Could you check a few things on this model? Use its own coordinates, in mm. Coordinates: 2 decimals unless noted, no trailing zeros. Write each loop counter-clockwise with the first axis right and the second up, starting at its lowest first coordinate (ties: lowest second). Pieces come first, ordered by that corner, then holes.
```python
from build123d import *

# Parameters (mm, degrees)
SKETCH_1_R          = 7.646875
EXTRUDE_555_DEPTH   = 17
SKETCH_2_OUTSIDE_W  = 129.344
SKETCH_2_OUTSIDE_H  = 133.304
SKETCH_2_OUTSIDE_R  = 13.5
CUT_EXTRUDE_1_DEPTH = 26.909162472
CUT_EXTRUDE_1_DRAFT = -60
CHAMFER_1_SIZE      = 0.294642857
SKETCH_9_OUTSIDE_W  = 89.946
SKETCH_9_OUTSIDE_H  = 93.906
SKETCH_9_OUTSIDE_R  = 12.15
CUT_EXTRUDE_7_DEPTH = 26.909162472
CUT_EXTRUDE_7_DRAFT = -45


with BuildPart() as part:
    # 草图1 → Extrude 555 (new body)
    with BuildSketch(Plane.XY):
        Polygon((0, 14.78), (-12.799855468, 7.39), (-12.799855468, -7.39), (0, -14.78), (12.799855468, -7.39), (12.799855468, 7.39), align=None)
        Circle(SKETCH_1_R, mode=Mode.SUBTRACT)
    extrude(amount=EXTRUDE_555_DEPTH)


with BuildPart() as cut_extrude_1_tool:
    # 草图2 outside → 切除-拉伸1 (with draft: the straight prism first)
    with BuildSketch(Plane(origin=(0, 0, 0), x_dir=(-1, 0, 0), z_dir=(0, 0, -1))):
        Rectangle(SKETCH_2_OUTSIDE_W, SKETCH_2_OUTSIDE_H)
        Circle(SKETCH_2_OUTSIDE_R, mode=Mode.SUBTRACT)
    extrude(amount=-CUT_EXTRUDE_1_DEPTH)
    # 切除-拉伸1: the draft: its side faces are tilted about the plane it starts from
    cut_extrude_1_sides = [cut_extrude_1_tool.faces().sort_by_distance(p)[0] for p in [
        (0, -66.652, 13.454581236),
        (-64.672, 0, 13.454581236),
        (0, 66.652, 13.454581236),
        (64.672, 0, 13.454581236),
        (13.5, 0, 13.454581236),
    ]]
    draft(cut_extrude_1_sides, Plane(origin=(0, 0, 0), x_dir=(-1, 0, 0), z_dir=(0, 0, -1)), CUT_EXTRUDE_1_DRAFT)


with BuildPart() as part_1:
    add(part.part)

    # 切除-拉伸1: cut by cut_extrude_1_tool
    add(cut_extrude_1_tool.part, mode=Mode.SUBTRACT)

    # 倒角1
    chamfer_1_edges = [part_1.edges().sort_by_distance(p)[0] for p in [
        (-7.646875, 0, 0),
    ]]
    chamfer(chamfer_1_edges, length=CHAMFER_1_SIZE)


with BuildPart() as cut_extrude_7_tool:
    # 草图9 outside → 切除-拉伸7 (with draft: the straight prism first)
    with BuildSketch(Plane.XY.offset(17)):
        Rectangle(SKETCH_9_OUTSIDE_W, SKETCH_9_OUTSIDE_H)
        Circle(SKETCH_9_OUTSIDE_R, mode=Mode.SUBTRACT)
    extrude(amount=-CUT_EXTRUDE_7_DEPTH)
    # 切除-拉伸7: the draft: its side faces are tilted about the plane it starts from
    cut_extrude_7_sides = [cut_extrude_7_tool.faces().sort_by_distance(p)[0] for p in [
        (0, -46.953, 3.545418764),
        (44.973, 0, 3.545418764),
        (0, 46.953, 3.545418764),
        (-44.973, 0, 3.545418764),
        (-12.15, 0, 3.545418764),
    ]]
    draft(cut_extrude_7_sides, Plane.XY.offset(17), CUT_EXTRUDE_7_DRAFT)


with BuildPart() as part_2:
    add(part_1.part)

    # 切除-拉伸7: cut by cut_extrude_7_tool
    add(cut_extrude_7_tool.part, mode=Mode.SUBTRACT)


solid = part_2.part
```
Item 1: If we mould it in two halves opening along Y, with no side actions, what happens to faces 1 (the flat face through (6.49, 11.033, 8.061)), 2 (the flat face through (-12.8, 0, 8)), 3 (the conical face through (-11.97, -6.96, 0.2)), 4 (the cylindrical face through (-5.636, 5.168, 8.53))? For each: released by +Y, released by -Y, zero draft, split by the parting line, or undercut.
Item 2: If I drill on line 1 along X through (y, z) = (-0.75, 4.5); line 2 along Y through (x, z) = (5.75, 11); line 3 along X through (y, z) = (1.5, 12), over which ranges is the centre line in solid material (lowest first)?
Item 3: Will this pin go through, and if not, where does the flat tip stop? pin 1 Ø1 at (x, z) = (6, 6.5) entering from +Y.
Item 4: I want a section at B-B, the plane z = 7.5. List the corners of the cut face in (x, y) for me.
Item 5: I want a section at A-A, the plane y = 0. List the corners of the cut face in (x, z) for me, then the cut area to 3 significant figures.
Taken from the geometry:
1. face 1: released by +Y
1. face 2: zero draft
1. face 3: released by -Y
1. face 4: undercut
2. line 1: x = -12.8 to -7.61, 7.61 to 12.8
2. line 2: y = -11.46 to -5.04, 5.04 to 11.46
2. line 3: x = -12.8 to -7.5, 7.5 to 12.8
3. pin 1: stops at y = 11.6
4. outline: (-12.8, -7.39) - (0, -14.78) - (12.8, -7.39) - (12.8, 7.39) - (0, 14.78) - (-12.8, 7.39) - close; hole circle Ø15.29 at (0, 0)
5. outline: (-12.8, 0) - (-7.94, 0) - (-7.65, 0.29) - (-7.65, 17) - (-12.15, 17) - (-12.8, 16.35) - close; (7.65, 0.29) - (7.94, 0) - (12.8, 0) - (12.8, 16.35) - (12.15, 17) - (7.65, 17) - close
5. area: 175 mm2
